Verification items for this drawing (mm, ordinates from the low corner). A direction names the side the tool comes from. Give positions to 0.01 mm unless a question says otherwise; leave off trailing zeros. Loops run counter-clockwise (first coordinate to the right, second up) from the corner with the lowest first, then second, coordinate; pieces in that order, holes last. Notation, with made-up numbers: (85, 29.25) -> (94, 29.25) arc R31 ccw to (94, 62.25) -> close; hole circle Ø5 at (44, 26). An arc over 180 degrees is marked (long way). Use one line per item in the form item = value. Start each with the question number.
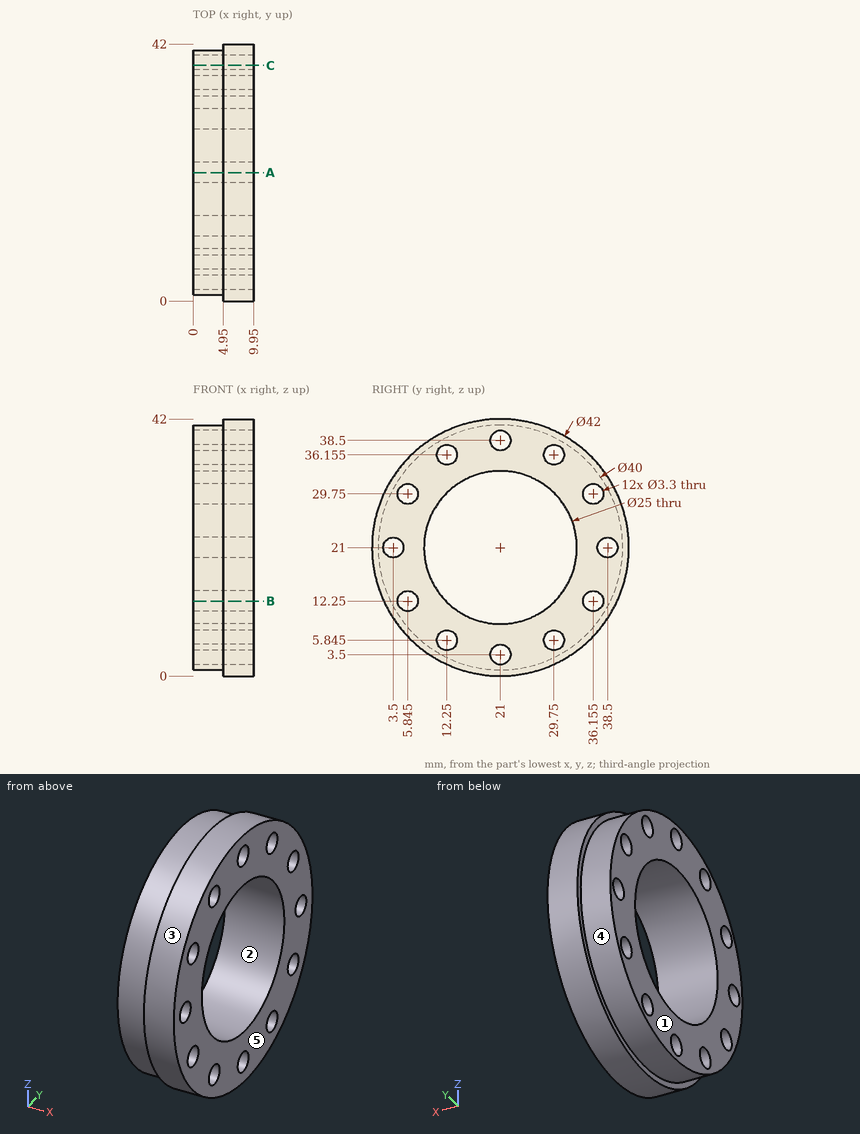
Item 1: Gauge pin test, flat ends, axial feed: pin 1 Ø1 at (x, z) = (5, 33) entering from +Y; pin 2 Ø2 at (y, z) = (12.25, 5.84) entering from -X; pin 3 Ø1 at (y, z) = (35, 36.5) entering from -X; pin 4 Ø3 at (x, y) = (3, 7) entering from +Z. Record the tip position at first contact, or that the pin passes through.
Item 2: Material ranges on line 1 (Y direction, x = 7.5, z = 12.5) (1 decimal); line 2 (Y direction, x = 4.25, z = 28.5) (1 decimal); line 3 (Z direction, x = 7.75, y = 36) (1 decimal), recorded low to high.
Item 3: Sectioned sample at A-A, the plane y = 21. Enter the section's corners in (x, z).
Item 4: Sectioned sample at B-B, the plane z = 12.25. State how many separate pieces and enclosed holes the cut face has, and give its area (3 significant figures).
Item 5: Draft check along Y on the marked faces 1, 2 and 3. Enter one of: +Y half, -Y half, draft (parallel to the pull), parting line (faces both ways), or undercut.
Item 6: Sectioned sample at C-C, the plane y = 38.5. Enter the section's corners in (x, z).
Item 7: Tool access check on the marked faces 4 and 5. Record the directions out of +Z, -Z, +X, -X, +Y, -Y that give a thin tool (end or side, any length) a straight path to the whole face; none if there is none.
Outcome:
q1.pin_1 = 38.57
q1.pin_2 = through
q1.pin_3 = 4.95
q1.pin_4 = 36.61
q2.line_1 = 1.8 to 4.2, 7.5 to 11.8, 30.2 to 34.5, 37.8 to 40.2
q2.line_2 = 2.5 to 4.8, 6.9 to 11, 31 to 35.1, 37.2 to 39.5
q2.line_3 = 6.3 to 10.6, 13.9 to 28.1, 31.4 to 35.7
q3.outline = (0, 1) -> (4.95, 1) -> (4.95, 0) -> (9.95, 0) -> (9.95, 1.85) -> (0, 1.85) -> close; (0, 5.15) -> (9.95, 5.15) -> (9.95, 8.5) -> (0, 8.5) -> close; (0, 33.5) -> (9.95, 33.5) -> (9.95, 36.85) -> (0, 36.85) -> close; (0, 40.15) -> (9.95, 40.15) -> (9.95, 42) -> (4.95, 42) -> (4.95, 41) -> (0, 41) -> close
q4.separate_pieces = 4
q4.enclosed_holes = 0
q4.area = 126 mm^2
q5.face_1 = draft
q5.face_2 = undercut
q5.face_3 = parting line
q6.outline = (0, 11.32) -> (4.95, 11.32) -> (4.95, 9.39) -> (9.95, 9.39) -> (9.95, 19.35) -> (0, 19.35) -> close; (0, 22.65) -> (9.95, 22.65) -> (9.95, 32.61) -> (4.95, 32.61) -> (4.95, 30.68) -> (0, 30.68) -> close
q7.face_4 = -X
q7.face_5 = +Z, -Z, +X, +Y, -Y
